```python
from build123d import *

# Parameters (mm, degrees)
EXTRUDE_1_DEPTH     = 50
CHAMFER_1_SIZE      = 3
CUT_EXTRUDE_1_REACH = 148.206
SKETCH_4_R          = 35.5


with BuildPart() as part:
    # 草图2 → 凸台-拉伸1 (new, symmetric)
    with BuildSketch(Plane(origin=(409.637600706, 0.5, -34.379468655), x_dir=(1, 0, 0), z_dir=(0, 0, 1))):
        Polygon((-409.637600706, 112), (-409.637600706, -0.5), (-457.637600706, -0.5), (-457.637600706, 7.5), (-417.637600706, 7.5), (-417.637600706, 112), align=None)
    extrude(amount=EXTRUDE_1_DEPTH, both=True)

    # 倒角1
    chamfer_1_edges = [part.edges().sort_by_distance(p)[0] for p in [
        (-48, 4, 15.620531345),
        (-4, 112.5, 15.620531345),
        (-48, 4, -84.379468655),
        (-4, 112.5, -84.379468655),
    ]]
    chamfer(chamfer_1_edges, length=CHAMFER_1_SIZE)

    # 草图4 → 切除-拉伸1 (cut, up to next)
    with BuildSketch(Plane.ZY.offset(8), mode=Mode.PRIVATE) as cut_extrude_1_sk1:
        with Locations((-34.379468655, 69.5)):
            Circle(SKETCH_4_R)
    cut_extrude_1_tool1 = extrude(cut_extrude_1_sk1.sketch, amount=-CUT_EXTRUDE_1_REACH, mode=Mode.PRIVATE) & part.part
    add(cut_extrude_1_tool1.solids().sort_by_distance((-8, 69.5, -34.379469))[0], mode=Mode.SUBTRACT)


solid = part.part
```
For this review, take the finished solid that the model builds, in its own axes (mm). A direction names the side the tool comes from. Give positions to 0.01 mm unless a question says otherwise; leave off trailing zeros. Order: outer loops, then holes, each group sorted by start corner. A loop starts at its lowest first (then second) coordinate and runs counter-clockwise, first axis right, second up.
1) Insertion check: pin 1 (6 mm diameter, centred on x = -31, z = -16.5, fed in from +Y); pin 2 (4 mm diameter, centred on y = 96, z = -6, fed in from -X). Each pin has a flat end and moves straight along its axis. Give the tip position at first contact, or say it passes through.
2) Wall thickness on line 1 (Z direction, x = -4, y = 69); line 2 (Y direction, x = -35, z = -64.5); line 3 (X direction, y = 24.5, z = -71): over which ranges is each line inside the solid? List them lowest first.
3) Take a section at D-D (z = -73). Give the boundary of the cut face in (x, y).
4) The part is to be moulded in two halves that separate along Z. For faces 1 (the face through (-4.1, 104.7, -39)), 2 (the face through (-7, 43, -84.379)), 3 (the face through (-48, 4, -34)), say which applies: released by +Z, released by -Z, zero draft, split by the parting line, or undercut.
5) For faces 4 (the face through (-4.06, 111.02, -82.86)), 5 (the face through (-8, 36, -11)), list the 3-axis set-ups (+Z, -Z, +X, -X, +Y, -Y) from which the entire face can be reached by the end or side of a thin tool; tool diameter is ignored.
6) Take a section at C-C (x = -5). Give the boundary of the cut face in (y, z).
7) Take a section at B-B (z = -40). Give the boundary of the cut face in (x, y).
8) Take a section at A-A (y = 69.5). Give the boundary of the cut face in (x, z).
Derived:
1. pin 1: stops at y = 8
1. pin 2: stops at x = -8
2. line 1: z = -84.38 to -69.88, 1.12 to 15.62
2. line 2: y = 0 to 8
2. line 3: x = -8 to 0
3. outline: (-48, 0) - (0, 0) - (0, 112.5) - (-8, 112.5) - (-8, 8) - (-48, 8) - close
4. face 1: undercut
4. face 2: released by -Z
4. face 3: zero draft
5. face 4: -Z, +X, -X, +Y
5. face 5: +Z, -Z, -X, +Y
6. outline: (0, -84.38) - (109.5, -84.38) - (112.5, -81.38) - (112.5, 12.62) - (109.5, 15.62) - (0, 15.62) - close; hole circle Ø71 at (69.5, -34.38)
7. outline: (-48, 0) - (0, 0) - (0, 34.45) - (-8, 34.45) - (-8, 8) - (-48, 8) - close; (-8, 104.55) - (0, 104.55) - (0, 112.5) - (-8, 112.5) - close
8. outline: (-8, -84.38) - (0, -84.38) - (0, -69.88) - (-8, -69.88) - close; (-8, 1.12) - (0, 1.12) - (0, 15.62) - (-8, 15.62) - close
